```python
from build123d import *

# Parameters (mm, degrees)
SKETCH1_R           = 19
BOSS_EXTRUDE1_DEPTH = 50
SKETCH2_R           = 32.5
BOSS_EXTRUDE2_DEPTH = 10
CUT_EXTRUDE1_REACH  = 69.915
SKETCH3_R           = 11.5
SKETCH4_R           = 3.5
CUT_EXTRUDE2_DEPTH  = 61.930288035
CIRPATTERN1_COUNT   = 4
CHAMFER1_SIZE       = 1
CHAMFER2_SIZE       = 2
CUT_EXTRUDE3_REACH  = 69.915


with BuildPart() as part:
    # Sketch1 → Boss-Extrude1 (new body)
    with BuildSketch(Plane(origin=(0, 0, 0), x_dir=(1, 0, 0), z_dir=(0, 1, 0))):
        with Locations(Location((0, 0, 0), (0, 0, 270))):
            Circle(SKETCH1_R)
    extrude(amount=BOSS_EXTRUDE1_DEPTH)

    # Sketch2 → Boss-Extrude2 (add)
    with BuildSketch(Plane(origin=(0, 50, 0), x_dir=(1, 0, 0), z_dir=(0, 1, 0))):
        with Locations(Location((0, 0, 0), (0, 0, 270))):
            Circle(SKETCH2_R)
    extrude(amount=-BOSS_EXTRUDE2_DEPTH)

    # Sketch3 → Cut-Extrude1 (cut, up to next)
    with BuildSketch(Plane.XZ, mode=Mode.PRIVATE) as cut_extrude1_sk1:
        with Locations(Location((0, 0, 0), (0, 0, 270))):
            Circle(SKETCH3_R)
    cut_extrude1_tool1 = extrude(cut_extrude1_sk1.sketch, amount=-CUT_EXTRUDE1_REACH, mode=Mode.PRIVATE) & part.part
    cut_extrude1 = cut_extrude1_tool1.solids().sort_by_distance((0, 0, 0))[0]
    add(cut_extrude1, mode=Mode.SUBTRACT)

    # Sketch4 → Cut-Extrude2 (cut, through all)
    with BuildSketch(Plane.XZ.offset(-40)):
        with Locations(Location((-27, 0, 0), (0, 0, 270))):
            Circle(SKETCH4_R)
    cut_extrude2 = extrude(amount=-CUT_EXTRUDE2_DEPTH, mode=Mode.SUBTRACT)

    # CirPattern1: Cut-Extrude1, Cut-Extrude2 ×4 about axis
    cirpattern1_axis = Axis((0, 0, 0), (0, 1, 0))
    add([cut_extrude1.rotate(cirpattern1_axis, i * 360 / CIRPATTERN1_COUNT) for i in range(1, CIRPATTERN1_COUNT)], mode=Mode.SUBTRACT)
    add([cut_extrude2.rotate(cirpattern1_axis, i * 360 / CIRPATTERN1_COUNT) for i in range(1, CIRPATTERN1_COUNT)], mode=Mode.SUBTRACT)

    # Chamfer1
    chamfer1_edges = [part.edges().sort_by_distance(p)[0] for p in [
        (0, 0, -19),
    ]]
    chamfer(chamfer1_edges, length=CHAMFER1_SIZE)

    # Chamfer2
    chamfer2_edges = [part.edges().sort_by_distance(p)[0] for p in [
        (0, 50, 11.5),
        (0, 0, 11.5),
    ]]
    chamfer(chamfer2_edges, length=CHAMFER2_SIZE)

    # Sketch5 → Cut-Extrude3 (cut, up to next)
    with BuildSketch(Plane(origin=(0, 50, 0), x_dir=(1, 0, 0), z_dir=(0, 1, 0)), mode=Mode.PRIVATE) as cut_extrude3_sk1:
        with BuildLine():
            Line((-25.617376915, -20), (25.617376915, -20))
            ThreePointArc((25.617376915, -20), (0, -32.5), (-25.617376915, -20))
        make_face()
    cut_extrude3_tool1 = extrude(cut_extrude3_sk1.sketch, amount=-CUT_EXTRUDE3_REACH, mode=Mode.PRIVATE) & part.part
    # Sketch5 → Cut-Extrude3 (cut, up to next)
    with BuildSketch(Plane(origin=(0, 50, 0), x_dir=(1, 0, 0), z_dir=(0, 1, 0)), mode=Mode.PRIVATE) as cut_extrude3_sk2:
        with BuildLine():
            Line((-25.617376915, 20), (25.617376915, 20))
            ThreePointArc((25.617376915, 20), (0, 32.5), (-25.617376915, 20))
        make_face()
    cut_extrude3_tool2 = extrude(cut_extrude3_sk2.sketch, amount=-CUT_EXTRUDE3_REACH, mode=Mode.PRIVATE) & part.part
    add(cut_extrude3_tool1.solids().sort_by_distance((0, 50, 25.09283))[0], mode=Mode.SUBTRACT)
    add(cut_extrude3_tool2.solids().sort_by_distance((0, 50, -25.09283))[0], mode=Mode.SUBTRACT)


solid = part.part
```
Can you work these out from the model? Positions are in its coordinate system, mm. A direction names the side the tool comes from. Give positions to 0.01 mm unless a question says otherwise; leave off trailing zeros. Order: outer loops, then holes, each group sorted by start corner. A loop starts at its lowest first (then second) coordinate and runs counter-clockwise, first axis right, second up. Notation, with made-up numbers: (72, 20.5) - (84, 20.5) arc R33 cw to (84, 51.5) - close; hole circle Ø10 at (84, -5). An arc over 180 degrees is marked (long way). Use a Markdown table: item, result. Add a question column.
Q1. If we section it at C-C on y = 32: Write out the boundary of the cut face in (x, z), plus the area to 3 significant figures.
Q2. If we mould it in two halves opening along Z, with no side actions, what happens to faces 3 (the cylindrical face through (23.53, 44.93, -0.46)), 4 (the flat face through (0, 45, 20)), 5 (the cylindrical face through (32.5, 45.1, 0.3)), 6 (the cylindrical face through (9.7, 24.68, -6.18))? For each: released by +Z, released by -Z, zero draft, split by the parting line, or undercut.
Q3. If we section it at B-B on x = 28.5: Write out the boundary of the cut face in (y, z), plus the area to 3 significant figures.
Q4. If we section it at A-A on z = 0: Write out the boundary of the cut face in (x, y), plus the area to 3 significant figures.
Q5. Please list where these lines run through material, in increasing order: line 1 along X through (y, z) = (43, 0); line 2 along X through (y, z) = (30, 0); line 3 along Y through (x, z) = (-11, -18).
Q6. I'm going to push flat-ended pins straight in: pin 1 (6 mm diameter, centred on x = -23.5, y = 14, fed in from +Z); pin 2 (2 mm diameter, centred on y = 15.5, z = -5, fed in from +X); pin 3 (1 mm diameter, centred on x = -2.5, y = 25.5, fed in from +Z); pin 4 (12 mm diameter, centred on y = 13.5, z = -9, fed in from +X). Where does each tip first touch, or does it pass through?
Q7. On a 3-axis mill with a long thin cutter (end or side, diameter ignored), from which of +Z, -Z, +X, -X, +Y, -Y can I reach the whole of each face in a straight line? I mean faces 1 (the conical face through (3.492, 48.125, -11.088)), 2 (the flat face through (8, 40, -18)). Say none if no direction works.
Answers follow:
| question | item | result |
|---|---|---|
| 1 | outline | circle Ø38 at (0, 0); hole circle Ø23 at (0, 0) |
| 1 | area | 719 mm^2 |
| 2 | face 3 | undercut |
| 2 | face 4 | released by +Z |
| 2 | face 5 | split by the parting line |
| 2 | face 6 | undercut |
| 3 | outline | (40, -15.62) - (50, -15.62) - (50, -3.16) - (40, -3.16) - close; (40, 3.16) - (50, 3.16) - (50, 15.62) - (40, 15.62) - close |
| 3 | area | 249 mm^2 |
| 4 | outline | (-32.5, 40) - (-30.5, 40) - (-30.5, 50) - (-32.5, 50) - close; (-23.5, 40) - (-19, 40) - (-19, 1) - (-18, 0) - (-13.5, 0) - (-11.5, 2) - (-11.5, 48) - (-13.5, 50) - (-23.5, 50) - close; (11.5, 2) - (13.5, 0) - (18, 0) - (19, 1) - (19, 40) - (23.5, 40) - (23.5, 50) - (13.5, 50) - (11.5, 48) - close; (30.5, 40) - (32.5, 40) - (32.5, 50) - (30.5, 50) - close |
| 4 | area | 871 mm^2 |
| 5 | line 1 | x = -32.5 to -30.5, -23.5 to -11.5, 11.5 to 23.5, 30.5 to 32.5 |
| 5 | line 2 | x = -19 to -11.5, 11.5 to 19 |
| 5 | line 3 | y = 40 to 50 |
| 6 | pin 1 | passes through |
| 6 | pin 2 | stops at x = 18.57 |
| 6 | pin 3 | stops at z = 18.89 |
| 6 | pin 4 | stops at x = 18.76 |
| 7 | face 1 | +Y |
| 7 | face 2 | -Y |
